Geometry: see drawing. Coordinates: mm, zero at the bounding-box minimum. Coordinates: 2 decimals unless noted, no trailing zeros. Write each loop counter-clockwise with the first axis right and the second up, starting at its lowest first coordinate (ties: lowest second). Pieces come first, ordered by that corner, then holes. Notation, with made-up numbers: (11.5, 22) - (67.5, 22) arc R24 cw to (67.5, 46) - close; hole circle Ø1 at (-12.5, -26.75). An arc over 180 degrees is marked (long way). One line per question, with ' | ' between items. Start each with the question number.
Q1. Cut plane A-A, the plane z = 7.75. Return loops of the section in (x, y) (1 decimal), plus the area to 3 significant figures.
Q2. Draft query along X for the marked faces 1, 2 and 3. Return one class per face: +X half, -X half, draft (parallel to the pull), parting line (faces both ways), or undercut.
Q3. Contact query for flat-ended pins moving along their axis: P1, Ø3, axis at y = 9.5, z = 5.5, coming from the +X side; P2, Ø6, axis at y = 2.5, z = 9, coming from the -X side (1 decimal); P3, Ø8, axis at y = 16.5, z = 6.5, coming from the -X side. Output: stop coordinate, or through.
Q4. Line query: line 1 (Y direction, x = 11.4, z = 9.5) (1 decimal); line 2 (X direction, y = 7.5, z = 1); line 3 (Y direction, x = 13.5, z = 1.25) (1 decimal). Output: solid intervals per line, ascending.
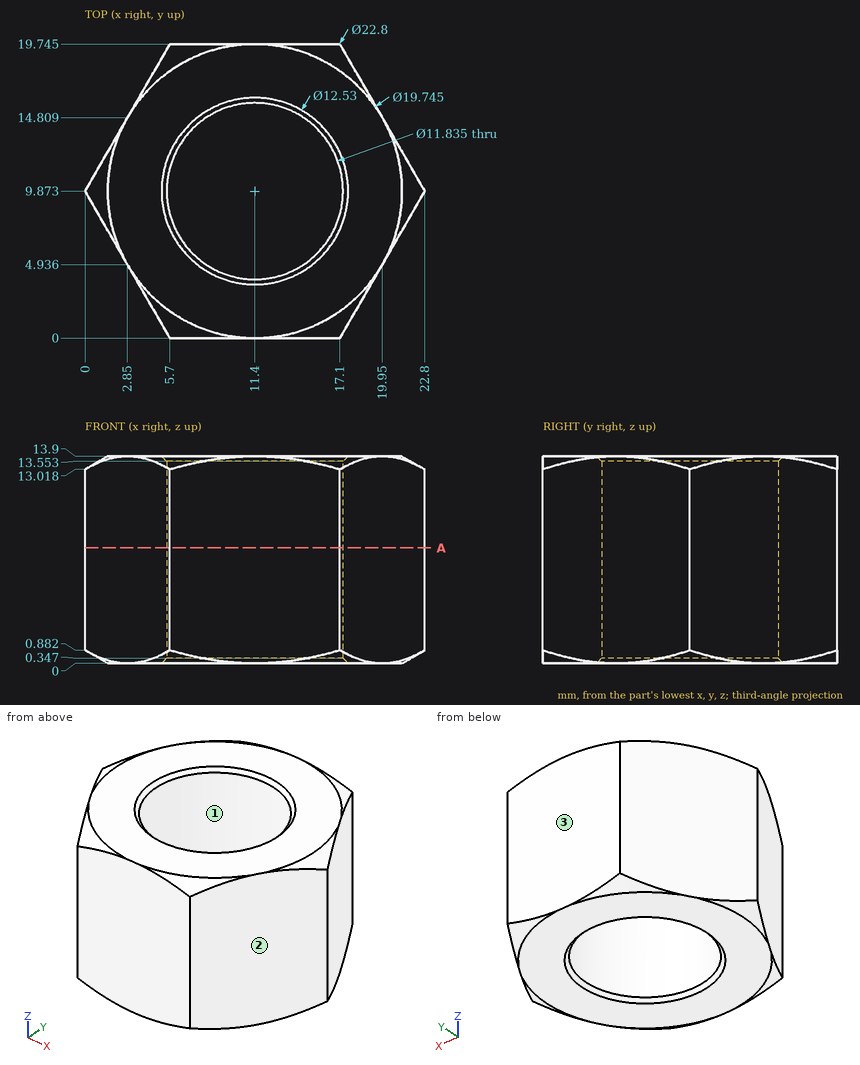
Reply:
1) outline: (0, 9.9) - (5.7, 0) - (17.1, 0) - (22.8, 9.9) - (17.1, 19.7) - (5.7, 19.7) - close; hole circle Ø11.8 at (11.4, 9.9) | area: 228 mm^2
2) face 1: undercut | face 2: +X half | face 3: draft
3) P1: stops at x = 22.8 | P2: stops at x = 2.5 | P3: stops at x = 1.52
4) line 1: y = 0 to 4, 15.8 to 19.7 | line 2: x = 1.37 to 5.98, 16.82 to 21.43 | line 3: y = 0 to 4.3, 15.4 to 19.7
